Geometry check sheet. Reference: the model listing, model coordinates, mm. A direction names the side the tool comes from. Give positions to 0.01 mm unless a question says otherwise; leave off trailing zeros. Order: outer loops, then holes, each group sorted by start corner. A loop starts at its lowest first (then second) coordinate and runs counter-clockwise, first axis right, second up. Notation, with made-up numbers: M -19.5,70 L -4.5,70 A16 ccw -4.5,81 Z; hole C 44.5,68 d10. An arc over 180 degrees is marked long. One line per question, with ' | ' between items. Start each with the question number.
from build123d import *

# Parameters (mm, degrees)
SKETCH1_W                                           = 44.75
SKETCH1_H                                           = 160
BOSS_EXTRUDE1_DEPTH                                 = 75
SKETCH5_W                                           = 34.75
SKETCH5_H                                           = 160
CUT_EXTRUDE3_DEPTH                                  = 20
F_8_5_8_5_DIAMETER_HOLE1_D                          = 8.5
CHAMFER2_SIZE                                       = 2
CBORE_FOR_M8_HEX_SOCKET_HEAD_CAP_SCREW1_D           = 9
CBORE_FOR_M8_HEX_SOCKET_HEAD_CAP_SCREW1_CBORE_D     = 15
CBORE_FOR_M8_HEX_SOCKET_HEAD_CAP_SCREW1_CBORE_DEPTH = 40


with BuildPart() as part:
    # Sketch1 → Boss-Extrude1 (new body)
    with BuildSketch(Plane(origin=(0, 0, 0), x_dir=(1, 0, 0), z_dir=(0, 1, 0))):
        Rectangle(SKETCH1_W, SKETCH1_H)
    extrude(amount=BOSS_EXTRUDE1_DEPTH)

    # Sketch5 → Cut-Extrude3 (cut)
    with BuildSketch(Plane.XZ):
        with Locations((5, 0)):
            Rectangle(SKETCH5_W, SKETCH5_H)
    extrude(amount=-CUT_EXTRUDE3_DEPTH, mode=Mode.SUBTRACT)

    # Ø8.5 (8.5) Diameter Hole1 (through all)
    with Locations(Plane(origin=(0, 75, 0), x_dir=(-1, 0, 0), z_dir=(0, 1, 0))):
        with Locations((-12.625, -60), (-12.625, 0), (-12.625, 60)):
            Hole(F_8_5_8_5_DIAMETER_HOLE1_D / 2)

    # Chamfer2
    chamfer2_edges = [part.edges().sort_by_distance(p)[0] for p in [
        (22.375, 47.5, 80),
        (-22.375, 37.5, 80),
        (-22.375, 37.5, -80),
        (22.375, 47.5, -80),
    ]]
    chamfer(chamfer2_edges, length=CHAMFER2_SIZE)

    # CBORE for M8 Hex Socket Head Cap Screw1 (through all)
    with Locations(Plane.XZ.offset(-20)):
        with Locations((12.625, 40), (12.625, -40)):
            CounterBoreHole(CBORE_FOR_M8_HEX_SOCKET_HEAD_CAP_SCREW1_D / 2, CBORE_FOR_M8_HEX_SOCKET_HEAD_CAP_SCREW1_CBORE_D / 2, CBORE_FOR_M8_HEX_SOCKET_HEAD_CAP_SCREW1_CBORE_DEPTH)


solid = part.part
Item 1: Depth check by flat-ended pin: pin 1 (16.5 mm diameter, centred on x = 15, z = -41, fed in from -Y); pin 2 (6 mm diameter, centred on y = 7.5, z = 27, fed in from +X) (3 decimals); pin 3 (11.5 mm diameter, centred on x = 12.625, z = 40, fed in from -Y); pin 4 (5 mm diameter, centred on x = 12.625, z = 60, fed in from +Y). Enter the tip coordinate at first touch or a pass-through.
Item 2: Material ranges on line 1 along Z through (x, y) = (9, 42.5); line 2 along Y through (x, z) = (16, 53); line 3 along Z through (x, y) = (6.5, 54), recorded low to high.
Item 3: Cross-section at A-A, the plane z = -40. Record the cut outline in (x, y) (3 decimals).
Item 4: Mould release check, pull along Z, two halves, no side actions. Record for faces 1 (the flat face through (-22.375, 37, 1)), 2 (the flat face through (0, 45, 80)), 3 (the flat face through (18, 60, -40)): released by +Z, released by -Z, zero draft, split by the parting line, or undercut.
Item 5: Cross-section at B-B, the plane y = 63.5. Record the cut outline in (x, z) (3 decimals).
Item 6: Set-up check for faces 4 (the cylindrical face through (11, 39.72, -47.32)), 5 (the flat face through (-12.375, 10, -1)), 6 (the cylindrical face through (10.549, 67.605, 36.008)): record each of +Z, -Z, +X, -X, +Y, -Y from which the full face is reachable in a straight line by a thin tool's end or side.
Item 7: Cross-section at C-C, the plane x = 14.5. State how many separate pieces and enclosed holes the cut face has, plus the area to 3 significant figures.
Item 8: Cross-section at D-D, the plane y = 43. Record the cut outline in (x, z) (3 decimals).
Outcome:
1) pin 1: stops at y = 20 | pin 2: stops at x = -12.375 | pin 3: stops at y = 60 | pin 4: passes through
2) line 1: z = -80 to -62.22, -57.78 to -46.57, -33.43 to -2.22, 2.22 to 33.43, 46.57 to 57.78, 62.22 to 80 | line 2: y = 20 to 75 | line 3: z = -80 to -44.33, -35.67 to 35.67, 44.33 to 80
3) outline: M -22.375,0 L -12.375,0 L -12.375,20 L 5.125,20 L 5.125,60 L 8.125,60 L 8.125,75 L -22.375,75 Z; M 17.125,60 L 20.125,60 L 20.125,20 L 22.375,20 L 22.375,75 L 17.125,75 Z
4) face 1: zero draft | face 2: released by +Z | face 3: undercut
5) outline: M -22.375,-78 L -20.375,-80 L 20.375,-80 L 22.375,-78 L 22.375,78 L 20.375,80 L -20.375,80 L -22.375,78 Z; hole C 12.625,-40 d9; hole C 12.625,40 d9; hole C 12.625,-60 d8.5; hole C 12.625,0 d8.5; hole C 12.625,60 d8.5
6) face 4: -Y | face 5: +Z, -Z, +X, -Y | face 6: +Y, -Y
7) separate pieces: 6 | enclosed holes: 0 | area: 6,130 mm²
8) outline: M -22.375,-78 L -20.375,-80 L 20.375,-80 L 22.375,-78 L 22.375,78 L 20.375,80 L -20.375,80 L -22.375,78 Z; hole C 12.625,-40 d15; hole C 12.625,40 d15; hole C 12.625,-60 d8.5; hole C 12.625,0 d8.5; hole C 12.625,60 d8.5
